Geometry check sheet. Reference: the model listing, model coordinates, mm. A direction names the side the tool comes from. Round coordinates to 2 decimals unless told otherwise and drop trailing zeros. Loops run counter-clockwise (first coordinate to the right, second up) from the corner with the lowest first, then second, coordinate; pieces in that order, holes last. Notation, with made-up numbers: (-38, 64.25) -> (7, 64.25) arc R29 cw to (7, 96.25) -> close; hole circle Ø7 at (32.25, -20.75). An arc over 180 degrees is marked (long way). Use a Markdown table: item, result. Add a question column.
Q1. Sectioned sample at C-C, the plane x = 0. Enter the section's corners in (y, z).
Q2. Gauge pin test, flat ends, axial feed: P1, Ø3, axis at y = 7, z = 20, coming from the -X side; P2, Ø1.6, axis at y = 2, z = 48, coming from the -X side; P3, Ø5, axis at y = 10.5, z = 37, coming from the +X side. Record the tip position at first contact, or that the pin passes through.
Q3. Sectioned sample at B-B, the plane x = -20.5. Enter the section's corners in (y, z).
Q4. Set-up check for faces 1 (the face through (-19, 3, -3)), 2 (the face through (19, 3, -1)), 3 (the face through (0.65, 9.57, -57.59)): record each of +Z, -Z, +X, -X, +Y, -Y from which the full face is reachable in a straight line by a thin tool's end or side.
Q5. Sectioned sample at A-A, the plane z = -40. Enter the section's corners in (x, y).
Q6. Release check for a two-part mould opening along Z. For faces 4 (the face through (0.65, 15.43, 55.41)), 5 (the face through (19, 1, 47)), 6 (the face through (22, 1.5, -40.9)) record: released by +Z, released by -Z, zero draft, split by the parting line, or undercut.
Q7. Material ranges on L1, parallel to X at y = 1.45, z = 40; L2, parallel to X at y = 4.75, z = 38.5; L3, parallel to Y at x = -17, z = -3, recorded low to high.
Q8. Sectioned sample at D-D, the plane z = 53.5. Enter the section's corners in (x, y), then the cut area to 3 significant figures.
```python
from build123d import *

# Parameters (mm, degrees)
EXTRUDE_1_DEPTH     = 100
SKETCH_2_W          = 98
SKETCH_2_H          = 3
EXTRUDE_2_DEPTH     = 10.6
SKETCH_3_W          = 2
SKETCH_3_H          = 6.4
CUT_EXTRUDE_1_DEPTH = 107.050978308
SKETCH_4_W          = 98
SKETCH_4_H          = 4.9
EXTRUDE_3_DEPTH     = 12.6
SKETCH_5_W          = 10.6
SKETCH_5_H          = 1.9
CUT_EXTRUDE_2_DEPTH = 107.050978308
SKETCH_6_R          = 3
EXTRUDE_4_DEPTH     = 13
EXTRUDE_START       = 13
SKETCH_7_R          = 3
EXTRUDE_5_DEPTH     = 13
SKETCH_10_R         = 1.75
CUT_EXTRUDE_3_DEPTH = 10


with BuildPart() as part:
    # 草图1 → 凸台-拉伸1 (new body)
    with BuildSketch(Plane.XY.offset(49)):
        with BuildLine():
            Line((-13.4, 0), (13.4, 0))
            Line((13.4, 0), (13.4, 12.5))
            ThreePointArc((13.4, 12.5), (0, 25.9), (-13.4, 12.5))
            Line((-13.4, 12.5), (-13.4, 0))
        make_face()
    extrude(amount=-EXTRUDE_1_DEPTH)

    # 草图2 → 凸台-拉伸2 (add)
    with BuildSketch(Plane(origin=(13.4, 0, 0), x_dir=(0, 0, -1), z_dir=(1, 0, 0))):
        with Locations((2, 1.5)):
            Rectangle(SKETCH_2_W, SKETCH_2_H)
    extrude(amount=EXTRUDE_2_DEPTH)

    # 草图3 → 切除-拉伸1 (cut, through all)
    with BuildSketch(Plane.XY.offset(49)):
        with Locations((-12.4, -0.2)):
            Rectangle(SKETCH_3_W, SKETCH_3_H)
    extrude(amount=-CUT_EXTRUDE_1_DEPTH, mode=Mode.SUBTRACT)

    # 草图4 → 凸台-拉伸3 (add)
    with BuildSketch(Plane.ZY.offset(11.4)):
        with Locations((-2, 2.45)):
            Rectangle(SKETCH_4_W, SKETCH_4_H)
    extrude(amount=EXTRUDE_3_DEPTH)

    # 草图5 → 切除-拉伸2 (cut, through all)
    with BuildSketch(Plane(origin=(0, 0, -51), x_dir=(-1, 0, 0), z_dir=(0, 0, -1))):
        with Locations((18.7, 3.95)):
            Rectangle(SKETCH_5_W, SKETCH_5_H)
    extrude(amount=-CUT_EXTRUDE_2_DEPTH, mode=Mode.SUBTRACT)

    # 草图6 → 凸台-拉伸4 (add)
    with BuildSketch(Plane.XY.offset(49)):
        with Locations(Location((0, 12.5, 0), (0, 0, 180))):
            Circle(SKETCH_6_R)
    extrude(amount=EXTRUDE_4_DEPTH)

    # 草图7 → 凸台-拉伸5 (add)
    with BuildSketch(Plane(origin=(0, 0, -51), x_dir=(-1, 0, 0), z_dir=(0, 0, -1)).offset(EXTRUDE_START)):
        with Locations((0, 12.5)):
            Circle(SKETCH_7_R)
    extrude(amount=-EXTRUDE_5_DEPTH)

    # 草图10 → 切除-拉伸3 (cut)
    with BuildSketch(Plane.XZ):
        with Locations(Location((-20.5, 40, 0), (0, 0, 270))):
            Circle(SKETCH_10_R)
        with Locations(Location((20.5, 40, 0), (0, 0, 270))):
            Circle(SKETCH_10_R)
        with Locations(Location((20.5, -40, 0), (0, 0, 270))):
            Circle(SKETCH_10_R)
        with Locations(Location((-20.5, -40, 0), (0, 0, 270))):
            Circle(SKETCH_10_R)
    extrude(amount=-CUT_EXTRUDE_3_DEPTH, mode=Mode.SUBTRACT)


solid = part.part
```
Values:
| question | item | result |
|---|---|---|
| 1 | outline | (0, -51) -> (9.5, -51) -> (9.5, -64) -> (15.5, -64) -> (15.5, -51) -> (25.9, -51) -> (25.9, 49) -> (15.5, 49) -> (15.5, 62) -> (9.5, 62) -> (9.5, 49) -> (0, 49) -> close |
| 2 | P1 | x = -13.4 |
| 2 | P2 | x = -11.4 |
| 2 | P3 | x = 13.4 |
| 3 | outline | (0, -51) -> (3, -51) -> (3, -41.75) -> (0, -41.75) -> close; (0, -38.25) -> (3, -38.25) -> (3, 38.25) -> (0, 38.25) -> close; (0, 41.75) -> (3, 41.75) -> (3, 47) -> (0, 47) -> close |
| 4 | face 1 | +Z, -Z, -X, +Y |
| 4 | face 2 | +Z, -Z, +X, +Y |
| 4 | face 3 | -Z |
| 5 | outline | (-24, 0) -> (-22.25, 0) -> (-22.25, 3) -> (-24, 3) -> close; (-18.75, 0) -> (18.75, 0) -> (18.75, 3) -> (13.4, 3) -> (13.4, 12.5) arc R13.4 ccw to (-13.4, 12.5) -> (-13.4, 3) -> (-18.75, 3) -> close; (22.25, 0) -> (24, 0) -> (24, 3) -> (22.25, 3) -> close |
| 6 | face 4 | zero draft |
| 6 | face 5 | released by +Z |
| 6 | face 6 | undercut |
| 7 | L1 | -24 to -22.25, -18.75 to 18.75, 22.25 to 24 |
| 7 | L2 | -13.4 to 13.4 |
| 7 | L3 | 0 to 3 |
| 8 | outline | circle Ø6 at (0, 12.5) |
| 8 | area | 28.3 mm^2 |
